Here's how the part is built. I have some questions about the finished solid (model axes, mm). A direction names the side the tool comes from. Coordinates: 2 decimals unless noted, no trailing zeros. Order: outer loops, then holes, each group sorted by start corner. A loop starts at its lowest first (then second) coordinate and runs counter-clockwise, first axis right, second up. Notation, with made-up numbers: (15, 51) - (46, 51) arc R26 cw to (46, 86) - close; hole circle Ø2 at (-21, 50.25). An arc over 180 degrees is marked (long way). Answer as CSV lines item,"result". Start each with the question number.
Q1. Suppose I cut it at B-B (y = 21). Please give me the cut outline in (x, z), then the cut area to 3 significant figures.
Q2. For faces 1 (the face through (2, 25, 6)), 2 (the face through (-1.802, 18.098, -5.723)), which set-ups out of +Z, -Z, +X, -X, +Y, -Y let a thin tool reach every point of the face, with its end or its side?
Q3. Thinking about a two-plate mould opening in Z: for faces 3 (the face through (6.668, 22.479, 8.696)), 4 (the face through (3, 0, -3)), 5 (the face through (3.92, 11, -1.42)), which applies, released by +Z, released by -Z, zero draft, split by the parting line, or undercut?
Q4. Suppose I cut it at A-A (y = 6.5). Please give me the cut outline in (x, z).
Q5. I need wall thicknesses on line 1 (X direction, y = 5, z = 0); line 2 (X direction, y = 20.25, z = 4.5); line 3 (Z direction, x = -5, y = 11.5). Which ranges of each line are inside material? Lowest first, please.
Q6. For pin 1 Ø12 at (y, z) = (16.5, -5) entering from +X; pin 2 Ø2 at (x, y) = (9.5, 6) entering from +Z; pin 3 Ø12 at (y, z) = (9.5, -8) entering from -X, each with a flat end and sliding along its axis, tell me the tip position at first contact or that it passes through.
from build123d import *


with BuildPart() as part:
    # Sketch1 → Revolve1 (revolve)
    with BuildSketch(Plane.XY, mode=Mode.PRIVATE) as revolve1_sk:
        with BuildLine():
            Line((4, 0), (4, 11))
            Line((4, 11), (6, 11))
            Line((6, 11), (6, 25))
            Line((6, 25), (9.310102051, 25))
            ThreePointArc((9.310102051, 25), (9.877970423, 24.823119379), (10.244948974, 24.355051026))
            Line((10.244948974, 24.355051026), (14.348469228, 13.550510257))
            ThreePointArc((14.348469228, 13.550510257), (14.835768711, 11.804897188), (15, 10))
            Line((15, 10), (15, 0))
            Line((15, 0), (4, 0))
        make_face()
    revolve(revolve1_sk.sketch.rotate(Axis((0, 0, 0), (0, 1, 0)), 90), axis=Axis((0, 0, 0), (0, 1, 0)))


solid = part.part
Here are the results:
1,outline,"circle Ø23.04 at (0, 0); hole circle Ø12 at (0, 0)"
1,area,"304 mm²"
2,face 1,"+Z, -Z, +X, -X, +Y"
2,face 2,"+Y"
3,face 3,"split by the parting line"
3,face 4,"zero draft"
3,face 5,"undercut"
4,outline,"circle Ø30 at (0, 0); hole circle Ø8 at (0, 0)"
5,line 1,"x = -15 to -4, 4 to 15"
5,line 2,"x = -10.91 to -3.97, 3.97 to 10.91"
5,line 3,"z = -14.02 to -3.32, 3.32 to 14.02"
6,pin 1,"stops at x = 14.79"
6,pin 2,"stops at z = 12.36"
6,pin 3,"stops at x = -14.87"
